```python
from build123d import *

# Parameters (mm, degrees)
SKETCH1_R           = 10
BOSS_EXTRUDE1_DEPTH = 6
SKETCH3_OUTSIDE_W   = 81.044
SKETCH3_OUTSIDE_H   = 83.318
SKETCH3_OUTSIDE_R   = 15.8
CUT_EXTRUDE2_DEPTH  = 10
CUT_EXTRUDE2_DRAFT  = -60
SKETCH4_OUTSIDE_W   = 63.722
SKETCH4_OUTSIDE_H   = 65.996
SKETCH4_OUTSIDE_R   = 15.8
CUT_EXTRUDE3_DEPTH  = 5
CUT_EXTRUDE3_DRAFT  = -60


with BuildPart() as part:
    # Sketch1 → Boss-Extrude1 (new body)
    with BuildSketch(Plane.XY):
        Polygon((-14.524594865, -11.417945408), (2.62593335, -18.287640837), (17.150528215, -6.869695429), (14.524594865, 11.417945408), (-2.62593335, 18.287640837), (-17.150528215, 6.869695429), align=None)
        Circle(SKETCH1_R, mode=Mode.SUBTRACT)
    extrude(amount=BOSS_EXTRUDE1_DEPTH)


with BuildPart() as cut_extrude2_tool:
    # Sketch3 outside → Cut-Extrude2 (with draft: the straight prism first)
    with BuildSketch(Plane.XY.offset(6)):
        Rectangle(SKETCH3_OUTSIDE_W, SKETCH3_OUTSIDE_H)
        Circle(SKETCH3_OUTSIDE_R, mode=Mode.SUBTRACT)
    extrude(amount=-CUT_EXTRUDE2_DEPTH)
    # Cut-Extrude2: the draft: its side faces are tilted about the plane it starts from
    cut_extrude2_sides = [cut_extrude2_tool.faces().sort_by_distance(p)[0] for p in [
        (0, -41.659, 1),
        (40.522, 0, 1),
        (0, 41.659, 1),
        (-40.522, 0, 1),
        (-15.8, 0, 1),
    ]]
    draft(cut_extrude2_sides, Plane.XY.offset(6), CUT_EXTRUDE2_DRAFT)


with BuildPart() as part_1:
    add(part.part)

    # Cut-Extrude2: cut by cut_extrude2_tool
    add(cut_extrude2_tool.part, mode=Mode.SUBTRACT)


with BuildPart() as cut_extrude3_tool:
    # Sketch4 outside → Cut-Extrude3 (with draft: the straight prism first)
    with BuildSketch(Plane(origin=(0, 0, 0), x_dir=(-1, 0, 0), z_dir=(0, 0, -1))):
        Rectangle(SKETCH4_OUTSIDE_W, SKETCH4_OUTSIDE_H)
        Circle(SKETCH4_OUTSIDE_R, mode=Mode.SUBTRACT)
    extrude(amount=-CUT_EXTRUDE3_DEPTH)
    # Cut-Extrude3: the draft: its side faces are tilted about the plane it starts from
    cut_extrude3_sides = [cut_extrude3_tool.faces().sort_by_distance(p)[0] for p in [
        (0, -32.998, 2.5),
        (-31.861, 0, 2.5),
        (0, 32.998, 2.5),
        (31.861, 0, 2.5),
        (15.8, 0, 2.5),
    ]]
    draft(cut_extrude3_sides, Plane(origin=(0, 0, 0), x_dir=(-1, 0, 0), z_dir=(0, 0, -1)), CUT_EXTRUDE3_DRAFT)


with BuildPart() as part_2:
    add(part_1.part)

    # Cut-Extrude3: cut by cut_extrude3_tool
    add(cut_extrude3_tool.part, mode=Mode.SUBTRACT)


solid = part_2.part
```
Geometry check sheet. Reference: the model listing, model coordinates, mm. Round coordinates to 2 decimals unless told otherwise and drop trailing zeros. Order: outer loops, then holes, each group sorted by start corner. A loop starts at its lowest first (then second) coordinate and runs counter-clockwise, first axis right, second up. Notation, with made-up numbers: (72, 70.5) - (127, 70.5) arc R29 cw to (127, 91.5) - close; hole circle Ø8 at (3.5, -29). An arc over 180 degrees is marked (long way). Use a Markdown table: item, result. Add a question column.
1) Section check B-B (z = 4). Record the cut outline in (x, y).
2) Section check A-A (y = 0). Record the cut outline in (x, z), then the cut area to 3 significant figures.
3) Gauge pin test, flat ends, axial feed: P1, Ø1.5, axis at x = 12.5, z = 3.5, coming from the +Y side; P2, Ø1.5, axis at y = 10.5, z = 1.5, coming from the +X side; P3, Ø3, axis at x = -8.5, z = 1.5, coming from the -Y side. Record the tip position at first contact, or that the pin passes through.
4) Mould release check, pull along Y, two halves, no side actions. Record for faces 1 (the cylindrical face through (-2.17, -9.76, 2.96)), 2 (the flat face through (-6.069, -14.805, 2.96)), 3 (the conical face through (-7.351, -14.133, 0.075)): released by +Y, released by -Y, zero draft, split by the parting line, or undercut.
5) Section check C-C (x = 0). Record the cut outline in (y, z), then the cut area to 3 significant figures.
6) Thickness scan on line 1 along X through (y, z) = (-9, 5.35); line 2 along Y through (x, z) = (0, 1.75); line 3 along X through (y, z) = (2.5, 4.15). Record the ranges inside material, lowest first.
Established:
| question | item | result |
|---|---|---|
| 1 | outline | (-17.15, 6.87) - (-14.52, -11.42) - (2.63, -18.29) - (17.15, -6.87) - (14.52, 11.42) - (-2.63, 18.29) - close; hole circle Ø20 at (0, 0) |
| 2 | outline | (-16.16, 0.21) - (-15.8, 0) - (-10, 0) - (-10, 6) - (-15.8, 6) - (-16.16, 5.79) - close; (10, 0) - (15.8, 0) - (16.16, 0.21) - (16.16, 5.79) - (15.8, 6) - (10, 6) - close |
| 2 | area | 73.8 mm2 |
| 3 | P1 | y = 12.53 |
| 3 | P2 | x = 14.76 |
| 3 | P3 | y = -14.43 |
| 4 | face 1 | undercut |
| 4 | face 2 | released by -Y |
| 4 | face 3 | split by the parting line |
| 5 | outline | (-17.24, 0.83) - (-15.8, 0) - (-10, 0) - (-10, 6) - (-15.8, 6) - (-17.24, 5.17) - close; (10, 0) - (15.8, 0) - (17.24, 0.83) - (17.24, 5.17) - (15.8, 6) - (10, 6) - close |
| 5 | area | 84.4 mm2 |
| 6 | line 1 | -14.33 to -4.36, 4.36 to 14.33 |
| 6 | line 2 | -17.24 to -10, 10 to 17.24 |
| 6 | line 3 | -16.52 to -9.68, 9.68 to 15.81 |
